```python
from build123d import *

# Parameters (mm, degrees)
BASE_BODY_DEPTH         = 30
SIDE_START              = -30
SIDE_POCKET_CUT_1_DEPTH = 18
SIDE_START_2            = 30
SIDE_POCKET_CUT_2_DEPTH = 18
SIDE_BLOCK_SKETCH_W     = 82
SIDE_BLOCK_SKETCH_H     = 35
SIDE_BLOCK_45X35_DEPTH  = 9
PIVOT_CYLINDER_SKETCH_R = 20
PIVOT_CYLINDER_40_DEPTH = 22
CYLINDER_SLOT_CUT_DEPTH = 12
PIVOT_BORE_SKETCH_R     = 8
PIVOT_BORE_16_DEPTH     = 9.99


with BuildPart() as part:
    # Base Profile Sketch → Base Body (new, symmetric)
    with BuildSketch(Plane(origin=(0, 0, 0), x_dir=(0, 0, -1), z_dir=(1, 0, 0))):
        Polygon((-45, 0), (45, 0), (25, 50), (0, 50), (-25, 50), align=None)
    extrude(amount=BASE_BODY_DEPTH, both=True)

    # Side Pocket Sketch → Side Pocket Cut 1 (cut)
    with BuildSketch(Plane(origin=(0, 0, 0), x_dir=(0, 0, -1), z_dir=(1, 0, 0)).offset(SIDE_START)):
        Polygon((-37, 20), (37, 20), (25, 50), (-25, 50), align=None)
    extrude(amount=SIDE_POCKET_CUT_1_DEPTH, mode=Mode.SUBTRACT)

    # Sketch5_2 → Side Pocket Cut 2 (cut)
    with BuildSketch(Plane(origin=(0, 0, 0), x_dir=(0, 0, -1), z_dir=(1, 0, 0)).offset(SIDE_START_2)):
        Polygon((-37, 20), (37, 20), (25, 50), (-25, 50), align=None)
    extrude(amount=-SIDE_POCKET_CUT_2_DEPTH, mode=Mode.SUBTRACT)

    # Side Block Sketch → Side Block 45x35 (add, symmetric)
    with BuildSketch(Plane(origin=(0, 0, 0), x_dir=(0, 0, -1), z_dir=(1, 0, 0))):
        with Locations((0, 27.5)):
            Rectangle(SIDE_BLOCK_SKETCH_W, SIDE_BLOCK_SKETCH_H)
    extrude(amount=SIDE_BLOCK_45X35_DEPTH, both=True)

    # Pivot Cylinder Sketch → Pivot Cylinder _40 (add, symmetric)
    with BuildSketch(Plane(origin=(0, 0, 0), x_dir=(0, 0, -1), z_dir=(1, 0, 0))):
        with Locations((0, 50)):
            Circle(PIVOT_CYLINDER_SKETCH_R)
    extrude(amount=PIVOT_CYLINDER_40_DEPTH, both=True)

    # Cylinder Slot Sketch → Cylinder Slot Cut (cut, symmetric)
    with BuildSketch(Plane(origin=(0, 0, 0), x_dir=(0, 0, -1), z_dir=(1, 0, 0))):
        with BuildLine():
            Line((-8, 68.33030278), (-8, 50))
            Line((-8, 50), (-20, 50))
            ThreePointArc((-20, 50), (-16.733200531, 60.95445115), (-8, 68.33030278))
        make_face()
    cylinder_slot_cut = extrude(amount=CYLINDER_SLOT_CUT_DEPTH, both=True, mode=Mode.SUBTRACT)

    # Cylinder Slot Mirror: Cylinder Slot Cut across plane
    add(cylinder_slot_cut.mirror(Plane.XY), mode=Mode.SUBTRACT)

    # Pivot Bore Sketch → Pivot Bore _16 (cut)
    with BuildSketch(Plane(origin=(22, 0, 0), x_dir=(0, 0, -1), z_dir=(1, 0, 0))):
        with Locations((0, 50)):
            Circle(PIVOT_BORE_SKETCH_R)
    pivot_bore_16 = extrude(amount=-PIVOT_BORE_16_DEPTH, mode=Mode.SUBTRACT)

    # Pivot Bore Mirror: Pivot Bore _16 across plane
    add(pivot_bore_16.mirror(Plane(origin=(0, 0, 0), x_dir=(0, 0, 1), z_dir=(1, 0, 0))), mode=Mode.SUBTRACT)


solid = part.part
```
Could you check a few things on this model? Use its own coordinates, in mm. A direction names the side the tool comes from. Round coordinates to 2 decimals unless told otherwise and drop trailing zeros. Loops run counter-clockwise (first coordinate to the right, second up) from the corner with the lowest first, then second, coordinate; pieces in that order, holes last. Notation, with made-up numbers: (56, 50) - (96, 50) arc R32 cw to (96, 78) - close; hole circle Ø2 at (-31.5, 14.5). An arc over 180 degrees is marked (long way). Answer as CSV lines item,"result".
1. On a 3-axis mill with a long thin cutter (end or side, diameter ignored), from which of +Z, -Z, +X, -X, +Y, -Y can I reach the whole of each face in a straight line? I mean faces 1 (the face through (-9, 36, -37)), 2 (the face through (-12.01, 50, 0)), 3 (the face through (0, 27, -41)). Say none if no direction works.
Filled in:
face 1,"-Z, -X, +Y"
face 2,"-X"
face 3,"-Z, +X, -X, +Y"
2. We'd pull the mould along Y, two halves only. Please class faces 4 (the face through (0, 50, -16)), 5 (the face through (-22, 41, 0)), 6 (the face through (0.31, 69.83, 2.6)), 7 (the face through (21, 20, 1)): +Y half, -Y half, draft (parallel to the pull), parting line (faces both ways), or undercut.
Filled in:
face 4,"+Y half"
face 5,"draft"
face 6,"undercut"
face 7,"undercut"
3. I want a section at C-C on x = 3. List the corners of the cut face in (y, z) for me.
Filled in:
outline,"(0, -45) - (10, -41) - (45, -41) - (45, -27) - (50, -25) - (50, -8) - (68.33, -8) arc R20 ccw to (68.33, 8) - (50, 8) - (50, 25) - (45, 27) - (45, 41) - (10, 41) - (0, 45) - close"
4. Please list where these lines run through material, in increasing order: line 1 along Y through (x, z) = (-14, 0); line 2 along Z through (x, y) = (8, 58.5); line 3 along Y through (x, z) = (13, 29). Write a range as [from, to].
Filled in:
line 1,"y = [0, 20], [30, 42], [58, 70]"
line 2,"z = [-8, 8]"
line 3,"y = [0, 20]"
5. I want a section at B-B on z = 16. List the corners of the cut face in (x, y) for me, then the cut area to 3 significant figures.
Filled in:
outline,"(-30, 0) - (30, 0) - (30, 20) - (12, 20) - (12, 38) - (22, 38) - (22, 62) - (12, 62) - (12, 50) - (-12, 50) - (-12, 62) - (-22, 62) - (-22, 38) - (-12, 38) - (-12, 20) - (-30, 20) - close"
area,"2,400 mm^2"
6. I want a section at A-A on y = 34. List the corners of the cut face in (x, z) for me.
Filled in:
outline,"(-22, -12) - (-12, -12) - (-12, -31.4) - (-9, -31.4) - (-9, -41) - (9, -41) - (9, -31.4) - (12, -31.4) - (12, -12) - (22, -12) - (22, 12) - (12, 12) - (12, 31.4) - (9, 31.4) - (9, 41) - (-9, 41) - (-9, 31.4) - (-12, 31.4) - (-12, 12) - (-22, 12) - close"
7. For pin 1 Ø15.5 at (y, z) = (30.5, 31.5) entering from -X; pin 2 Ø14.5 at (x, y) = (4.5, 20.5) entering from +Z; pin 3 Ø8.5 at (x, z) = (4.5, 18) entering from +Y, each with a flat end and sliding along its axis, tell me the tip position at first contact or that it passes through.
Filled in:
pin 1,"stops at x = -12"
pin 2,"stops at z = 41"
pin 3,"stops at y = 50"
8. I want a section at D-D on z = 0. List the corners of the cut face in (x, y) for me.
Filled in:
outline,"(-30, 0) - (30, 0) - (30, 20) - (12, 20) - (12, 30) - (22, 30) - (22, 42) - (12.01, 42) - (12.01, 58) - (22, 58) - (22, 70) - (-22, 70) - (-22, 58) - (-12.01, 58) - (-12.01, 42) - (-22, 42) - (-22, 30) - (-12, 30) - (-12, 20) - (-30, 20) - close"
